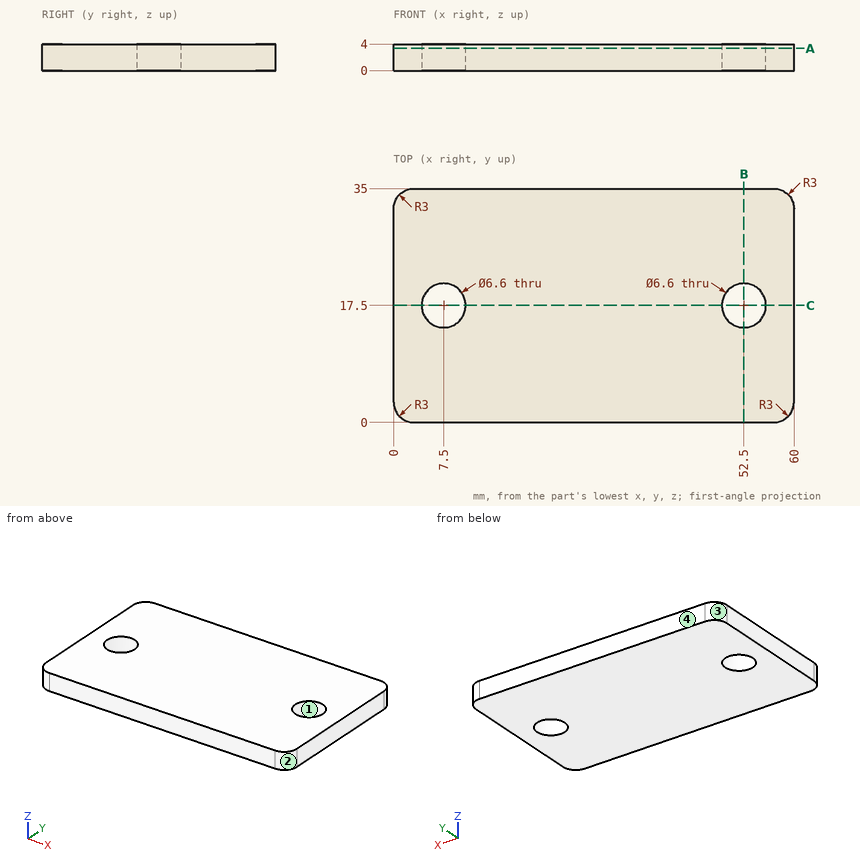
The drawing under review shows one solid part. Ordinate dimensions are in mm from its lowest x, y, z. Round coordinates to 2 decimals unless told otherwise and drop trailing zeros. Loops run counter-clockwise (first coordinate to the right, second up) from the corner with the lowest first, then second, coordinate; pieces in that order, holes last. Notation, with made-up numbers: (-9.75, -11.5) - (38.25, -11.5) arc R17 cw to (38.25, 10.5) - close; hole circle Ø7 at (-9, 54). An arc over 180 degrees is marked (long way). Use a Markdown table: item, result. Add a question column.
Q1. Add section C-C (y = 17.5). State the section outline as (x, z) points, plus the area to 3 significant figures.
Q2. Insertion check: pin 1 Ø6 at (x, y) = (7.5, 16.5) entering from -Z. The pin has a flat end and moves straight along its axis. Give the tip position at first contact, or say it passes through.
Q3. For probe 1 along Y at (x, z) = (52.5, 2.15); probe 2 along X at (y, z) = (18.5, 0.5); probe 3 along X at (y, z) = (19.5, 2.85), list the stretches that pass through material, from the lowest coordinate up.
Q4. Add section A-A (z = 3.35). State the section outline as (x, y) points, plus the area to 3 significant figures.
Q5. Add section B-B (x = 52.5). State the section outline as (y, z) points.
Q6. The part is to be moulded in two halves that separate along X. For the marked faces 1, 2, 3 and 4, say which applies: pulls with the +X half, pulls with the -X half, needs draft (parallel to the pull), parting line crosses it, or undercut.
Worked answers:
| question | item | result |
|---|---|---|
| 1 | outline | (0, 0) - (4.2, 0) - (4.2, 4) - (0, 4) - close; (10.8, 0) - (49.2, 0) - (49.2, 4) - (10.8, 4) - close; (55.8, 0) - (60, 0) - (60, 4) - (55.8, 4) - close |
| 1 | area | 187 mm² |
| 2 | pin 1 | z = 0 |
| 3 | probe 1 | 0 to 14.2, 20.8 to 35 |
| 3 | probe 2 | 0 to 4.36, 10.64 to 49.36, 55.64 to 60 |
| 3 | probe 3 | 0 to 4.88, 10.12 to 49.88, 55.12 to 60 |
| 4 | outline | (0, 3) arc R3 ccw to (3, 0) - (57, 0) arc R3 ccw to (60, 3) - (60, 32) arc R3 ccw to (57, 35) - (3, 35) arc R3 ccw to (0, 32) - close; hole circle Ø6.6 at (7.5, 17.5); hole circle Ø6.6 at (52.5, 17.5) |
| 4 | area | 2,020 mm² |
| 5 | outline | (0, 0) - (14.2, 0) - (14.2, 4) - (0, 4) - close; (20.8, 0) - (35, 0) - (35, 4) - (20.8, 4) - close |
| 6 | face 1 | undercut |
| 6 | face 2 | pulls with the +X half |
| 6 | face 3 | pulls with the -X half |
| 6 | face 4 | needs draft |
